Print and shaded views of the part. All mm, measured from the part's lowest x, y and z. A direction names the side the tool comes from. Give positions to 0.01 mm unless a question says otherwise; leave off trailing zeros. Write each loop counter-clockwise with the first axis right and the second up, starting at its lowest first coordinate (ties: lowest second). Pieces come first, ordered by that corner, then holes. Notation, with made-up numbers: (-31.5, 54) -> (-23.5, 54) arc R22 cw to (-23.5, 67) -> close; hole circle Ø4 at (-20, 23). An arc over 180 degrees is marked (long way). Put each result on its own line as item: value.
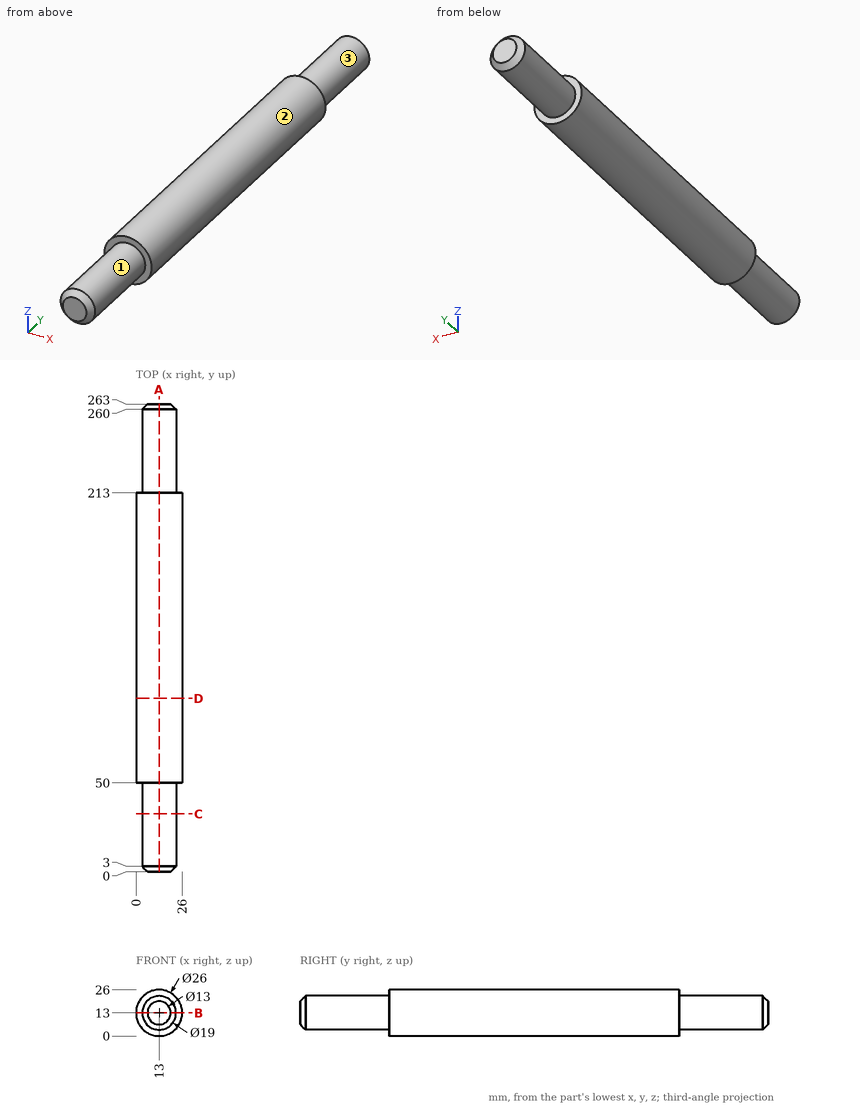
1) Tool access for the marked faces 1, 2 and 3: list every direction of +Z, -Z, +X, -X, +Y, -Y with a clear straight run to the whole face (end or side of a thin tool).
Filled sheet:
face 1: -Y
face 2: +Y, -Y
face 3: +Y
2) Pin check, flat tips, straight feed: pin 1 (12 mm diameter, centred on x = 20.5, y = 207.5, fed in from +Z); pin 2 (10 mm diameter, centred on x = 4, y = 64.5, fed in from -Z); pin 3 (1.5 mm diameter, centred on y = 55, z = 21, fed in from -X). Stop position of each tip, or through.
Filled sheet:
pin 1: z = 25.91
pin 2: z = 0.63
pin 3: x = 2.21
3) Slice it at C-C (y = 32.5). Write the cut outline in (x, z).
Filled sheet:
outline: circle Ø19 at (13, 13)
4) Slice it at D-D (y = 97.5). Write the cut outline in (x, z).
Filled sheet:
outline: circle Ø26 at (13, 13)
5) Wall check: L1, parallel to Z at x = 12.25, y = 72.5; L2, parallel to X at y = 69, z = 13.5; L3, parallel to Z at x = 12.5, y = 48.5. Give the ranges that are in metal, low to high.
Filled sheet:
L1: 0.02 to 25.98
L2: 0.01 to 25.99
L3: 3.51 to 22.49
6) Slice it at B-B (z = 13). Write the cut outline in (x, y).
Filled sheet:
outline: (0, 50) -> (3.5, 50) -> (3.5, 3) -> (6.5, 0) -> (19.5, 0) -> (22.5, 3) -> (22.5, 50) -> (26, 50) -> (26, 213) -> (22.5, 213) -> (22.5, 260) -> (19.5, 263) -> (6.5, 263) -> (3.5, 260) -> (3.5, 213) -> (0, 213) -> close
7) Slice it at A-A (x = 13). Write the cut outline in (y, z).
Filled sheet:
outline: (0, 6.5) -> (3, 3.5) -> (50, 3.5) -> (50, 0) -> (213, 0) -> (213, 3.5) -> (260, 3.5) -> (263, 6.5) -> (263, 19.5) -> (260, 22.5) -> (213, 22.5) -> (213, 26) -> (50, 26) -> (50, 22.5) -> (3, 22.5) -> (0, 19.5) -> close
